Design review of the part built by this model. Coordinates are the model's own, in mm. Face numbers are marked on the shaded views. A direction names the side the tool comes from. Coordinates: 2 decimals unless noted, no trailing zeros. Loops run counter-clockwise (first coordinate to the right, second up) from the corner with the lowest first, then second, coordinate; pieces in that order, holes last. Notation, with made-up numbers: (75, -0.75) -> (128, -0.75) arc R32 cw to (128, 33.25) -> close; hole circle Ø11 at (61, -18). An arc over 180 degrees is marked (long way). Use a Markdown table: item, result. Add a question column.
Q1. Take a section at D-D on x = 45. Write out the cut boundary in (y, z), plus the area to 3 significant figures.
Q2. Clearance check with flat-ended pins moving along their axes: pin 1 Ø2.5 at (x, z) = (5, 176.5) entering from -Y; pin 2 Ø21 at (x, z) = (38.5, 33) entering from +Y; pin 3 Ø6.5 at (y, z) = (5.5, 25.5) entering from -X. State where each tip first meets the part, or that it passes through.
Q3. Take a section at C-C on z = 50. Write out the cut boundary in (x, y).
Q4. Take a section at A-A on x = 30. Write out the cut boundary in (y, z).
Q5. For the marked faces 1 and 2, list the 3-axis set-ups (+Z, -Z, +X, -X, +Y, -Y) from which the entire face can be reached by the end or side of a thin tool; tool diameter is ignored.
Q6. For probe 1 along Y at (x, z) = (4.5, 234); probe 2 along Y at (x, z) = (3, 85); probe 3 along X at (y, z) = (21.5, 63.5), list the stretches that pass through material, from the lowest coordinate up.
Q7. Draft analysis for pull direction X (two halves, no side actions). For the marked faces 3, 4 and 5, state which applies: pulls with the +X half, pulls with the -X half, needs draft (parallel to the pull), parting line crosses it, or undercut.
Q8. Take a section at B-B on y = 55. Write out the cut boundary in (x, z), plus the area to 3 significant figures.
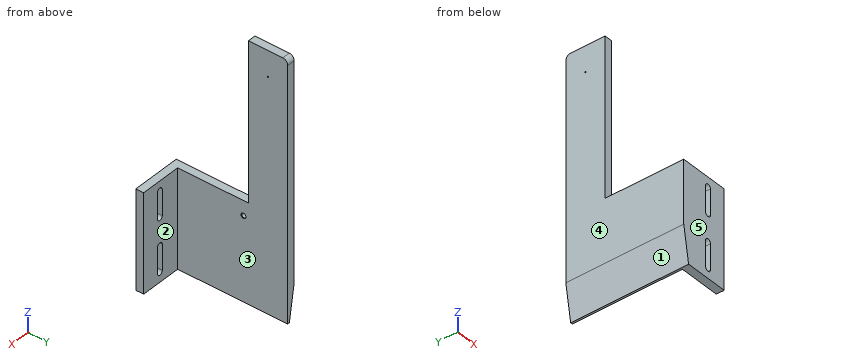
from build123d import *

# Parameters (mm, degrees)
BOSS_EXTRUDE1_DEPTH         = 260
SKETCH2_W                   = 160
SKETCH2_H                   = 80
CUT_EXTRUDE1_DEPTH          = 291.688837075
CUT_EXTRUDE2_DEPTH          = 220
CUT_EXTRUDE3_DEPTH          = 291.688837075
M5_TAPPED_HOLE1_D           = 4.2
M5_TAPPED_HOLE1_DEPTH       = 6
M5_TAPPED_HOLE1_CSINK_D     = 5.05
M5_TAPPED_HOLE1_CSINK_ANGLE = 90
M5_TAPPED_HOLE1_TIP         = 1.2618073
FILLET1_R                   = 5
SKETCH6_R                   = 0.6
CUT_EXTRUDE4_DEPTH          = 290.420109875


with BuildPart() as part:
    # Sketch1 → Boss-Extrude1 (new body)
    with BuildSketch(Plane.XY):
        Polygon((0, 0), (0, 120), (8, 120), (8, 8), (50, 8), (50, 0), align=None)
    extrude(amount=BOSS_EXTRUDE1_DEPTH)

    # Sketch2 → Cut-Extrude1 (cut, through all)
    with BuildSketch(Plane(origin=(50, 0, 0), x_dir=(0, 0, -1), z_dir=(1, 0, 0))):
        with Locations((-180, 40)):
            Rectangle(SKETCH2_W, SKETCH2_H)
    extrude(amount=-CUT_EXTRUDE1_DEPTH, mode=Mode.SUBTRACT)

    # Sketch3 → Cut-Extrude2 (cut)
    with BuildSketch(Plane(origin=(0, 8, 0), x_dir=(1, 0, 0), z_dir=(0, 1, 0))):
        with BuildLine():
            Line((27, -90), (27, -64))
            ThreePointArc((27, -64), (30, -61), (33, -64))
            Line((33, -64), (33, -90))
            ThreePointArc((33, -90), (30, -93), (27, -90))
        make_face()
        with BuildLine():
            Line((27, -36), (27, -10))
            ThreePointArc((27, -10), (30, -7), (33, -10))
            Line((33, -10), (33, -36))
            ThreePointArc((33, -36), (30, -39), (27, -36))
        make_face()
    extrude(amount=-CUT_EXTRUDE2_DEPTH, mode=Mode.SUBTRACT)

    # Sketch4 → Cut-Extrude3 (cut, through all)
    with BuildSketch(Plane(origin=(0, 120, 0), x_dir=(1, 0, 0), z_dir=(0, 1, 0))):
        Polygon((6, 0), (0, -36), (0, 0), align=None)
    extrude(amount=-CUT_EXTRUDE3_DEPTH, mode=Mode.SUBTRACT)

    # M5 Tapped Hole1
    with Locations(Plane(origin=(8, 75, 85), x_dir=(0, 0, 1), z_dir=(1, 0, 0))):
        with Locations((0, 0)):
            CounterSinkHole(M5_TAPPED_HOLE1_D / 2, M5_TAPPED_HOLE1_CSINK_D / 2, depth=M5_TAPPED_HOLE1_DEPTH, counter_sink_angle=M5_TAPPED_HOLE1_CSINK_ANGLE)
            with Locations((0, 0, -(M5_TAPPED_HOLE1_DEPTH + M5_TAPPED_HOLE1_TIP / 2))):  # 118° drill point
                Cone(0, M5_TAPPED_HOLE1_D / 2, M5_TAPPED_HOLE1_TIP, mode=Mode.SUBTRACT)

    # Fillet1
    fillet1_edges = [part.edges().sort_by_distance(p)[0] for p in [
        (4, 120, 260),
    ]]
    fillet(fillet1_edges, radius=FILLET1_R)

    # Sketch6 → Cut-Extrude4 (cut, through all)
    with BuildSketch(Plane(origin=(8, 0, 0), x_dir=(0, 0, -1), z_dir=(1, 0, 0))):
        with Locations((-234, 100)):
            Circle(SKETCH6_R)
    extrude(amount=-CUT_EXTRUDE4_DEPTH, mode=Mode.SUBTRACT)


solid = part.part
Answer list:
| question | item | result |
|---|---|---|
| 1 | outline | (0, 0) -> (8, 0) -> (8, 100) -> (0, 100) -> close |
| 1 | area | 800 mm² |
| 2 | pin 1 | y = 80 |
| 2 | pin 2 | y = 8 |
| 2 | pin 3 | x = 1.21 |
| 3 | outline | (0, 0) -> (50, 0) -> (50, 8) -> (8, 8) -> (8, 120) -> (0, 120) -> close |
| 4 | outline | (0, 0) -> (8, 0) -> (8, 7) -> (0, 7) -> close; (0, 39) -> (8, 39) -> (8, 61) -> (0, 61) -> close; (0, 93) -> (8, 93) -> (8, 100) -> (0, 100) -> close |
| 5 | face 1 | -Z, -X, +Y, -Y |
| 5 | face 2 | +Z, -Z, +X, +Y |
| 6 | probe 1 | 80 to 99.4, 100.6 to 120 |
| 6 | probe 2 | 0 to 72.9, 77.1 to 120 |
| 6 | probe 3 | 0 to 8 |
| 7 | face 3 | pulls with the +X half |
| 7 | face 4 | pulls with the -X half |
| 7 | face 5 | needs draft |
| 8 | outline | (0, 36) -> (6, 0) -> (8, 0) -> (8, 100) -> (0, 100) -> close |
| 8 | area | 692 mm² |
